The model under review builds one solid part; all positions refer to its coordinate system, in mm. Coordinates: 2 decimals unless noted, no trailing zeros. Order: outer loops, then holes, each group sorted by start corner. A loop starts at its lowest first (then second) coordinate and runs counter-clockwise, first axis right, second up. Notation, with made-up numbers: (25, -12.5) -> (63, -12.5) arc R13 ccw to (63, -0.5) -> close; hole circle Ø6 at (24.5, 71.5). An arc over 180 degrees is marked (long way). Use CSV: the item, a comma, the result in double quotes. Start each with the question number.
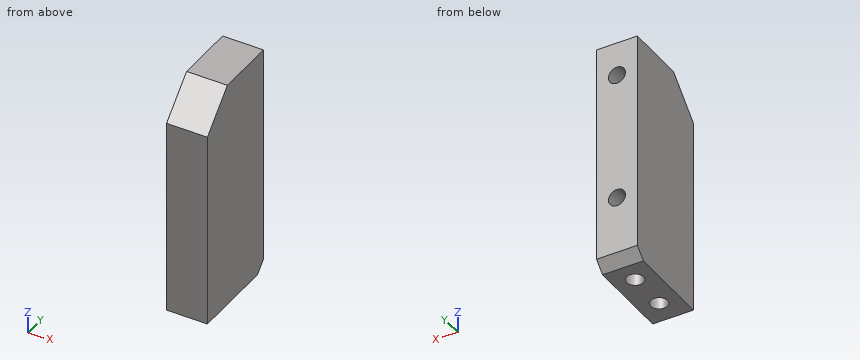
```python
from build123d import *

# Parameters (mm, degrees)
SKETCH_1_W             = 12
SKETCH_1_H             = 28
EXTRUDE_1_DEPTH        = 68
CHAMFER_1_SIZE         = 10
CHAMFER_2_SIZE         = 3
HOLE_WIZARD_M6_1_D     = 5
HOLE_WIZARD_M6_1_DEPTH = 13
HOLE_WIZARD_M6_1_TIP   = 1.502151548
HOLE_WIZARD_M6_2_D     = 5
HOLE_WIZARD_M6_2_DEPTH = 13
HOLE_WIZARD_M6_2_TIP   = 1.502151548


with BuildPart() as part:
    # 草图1 → 凸台-拉伸1 (new body)
    with BuildSketch(Plane.XY):
        with Locations((-244.955728906, -14)):
            Rectangle(SKETCH_1_W, SKETCH_1_H)
    extrude(amount=EXTRUDE_1_DEPTH)

    # 倒角1
    chamfer_1_edges = [part.edges().sort_by_distance(p)[0] for p in [
        (-244.955728906, -28, 68),
    ]]
    chamfer(chamfer_1_edges, length=CHAMFER_1_SIZE)

    # 倒角2
    chamfer_2_edges = [part.edges().sort_by_distance(p)[0] for p in [
        (-244.955728906, 0, 0),
    ]]
    chamfer(chamfer_2_edges, length=CHAMFER_2_SIZE)

    # M6 螺纹孔1
    with Locations(Plane(origin=(0, 0, 0), x_dir=(-1, 0, 0), z_dir=(0, 0, -1))):
        with Locations((244.955728906, -9), (244.955728906, -21)):
            Hole(HOLE_WIZARD_M6_1_D / 2, depth=HOLE_WIZARD_M6_1_DEPTH)
            with Locations((0, 0, -(HOLE_WIZARD_M6_1_DEPTH + HOLE_WIZARD_M6_1_TIP / 2))):  # 118° drill point
                Cone(0, HOLE_WIZARD_M6_1_D / 2, HOLE_WIZARD_M6_1_TIP, mode=Mode.SUBTRACT)

    # M6 螺纹孔2
    with Locations(Plane(origin=(0, 0, 0), x_dir=(1, 0, 0), z_dir=(0, 1, 0))):
        with Locations((-244.955728906, -58), (-244.955728906, -20)):
            Hole(HOLE_WIZARD_M6_2_D / 2, depth=HOLE_WIZARD_M6_2_DEPTH)
            with Locations((0, 0, -(HOLE_WIZARD_M6_2_DEPTH + HOLE_WIZARD_M6_2_TIP / 2))):  # 118° drill point
                Cone(0, HOLE_WIZARD_M6_2_D / 2, HOLE_WIZARD_M6_2_TIP, mode=Mode.SUBTRACT)


solid = part.part
```
Q1. Clearance check with flat-ended pins moving along their axes: pin 1 Ø1 at (x, y) = (-246.5, -20) entering from +Z; pin 2 Ø3 at (x, y) = (-244.96, -21) entering from -Z. State where each tip first meets the part, or that it passes through.
Q2. Add section A-A, the plane z = 8. State the section outline as (x, y) points.
Q3. To check wall thickness, follow probe 1 along Z at (x, y) = (-245, -3.75); probe 2 along X at (y, z) = (-8.5, 20); probe 3 along Z at (x, y) = (-245.75, -3.5). State the ranges of each line that lie inside material, in increasing order.
Q4. Add section B-B, the plane x = -241. State the section outline as (y, z) points, then the cut area to 3 significant figures.
Q5. Add section D-D, the plane y = -10.5. State how many separate pieces and enclosed holes the cut face has, then the cut area to 3 significant figures.
Q6. Add section C-C, the plane z = 63.5. State the section outline as (x, y) points.
Answer block:
1,pin 1,"stops at z = 66.5"
1,pin 2,"stops at z = 13.6"
2,outline,"(-250.96, -28) -> (-238.96, -28) -> (-238.96, 0) -> (-250.96, 0) -> close; hole circle Ø5 at (-244.96, -21); hole circle Ø5 at (-244.96, -9)"
3,probe 1,"z = 0 to 17.5, 22.5 to 55.5, 60.5 to 68"
3,probe 2,"x = -250.96 to -247.46, -242.46 to -238.96"
3,probe 3,"z = 0 to 17.63, 22.37 to 55.63, 60.37 to 68"
4,outline,"(-28, 0) -> (-3, 0) -> (0, 3) -> (0, 68) -> (-18, 68) -> (-28, 58) -> close"
4,area,"1,850 mm²"
5,separate pieces,"1"
5,enclosed holes,"2"
5,area,"723 mm²"
6,outline,"(-250.96, -22.5) -> (-238.96, -22.5) -> (-238.96, 0) -> (-250.96, 0) -> close"
